For this review, take the finished solid that the model builds, in its own axes (mm). A direction names the side the tool comes from. Round coordinates to 2 decimals unless told otherwise and drop trailing zeros. Loops run counter-clockwise (first coordinate to the right, second up) from the corner with the lowest first, then second, coordinate; pieces in that order, holes last.
1. Consider section A-A on x = -55. State the section outline as (y, z) points.
2. Draft analysis for pull direction X (two halves, no side actions). For faces 6 (the flat face through (-20, 49, 14)), 7 (the flat face through (35, 47, 13)), 8 (the flat face through (-52, 25, 4)), 9 (the flat face through (20, 49, 14)), state which applies: released by +X, released by -X, zero draft, split by the parting line, or undercut.
3. To check wall thickness, follow line 1 along X through (y, z) = (45, 27); line 2 along Y through (x, z) = (-54, 14.5); line 3 along Y through (x, z) = (-6, -13.5). State the ranges of each line that lie inside material, in increasing order.
4. Tool access review of faces 1 (the flat face through (1, 0, -10)), 2 (the flat face through (-35, 47, 13)), 3 (the flat face through (-60, 12, -24.27)), 4 (the flat face through (57, 25, 4)), 5 (the cylindrical face through (0.77, 14.79, -73.26)): name each direction out of +Z, -Z, +X, -X, +Y, -Y from which nothing blocks a thin tool from reaching the whole face with its end or side.
5. Clearance check with flat-ended pins moving along their axes: pin 1 Ø12 at (y, z) = (64, 2) entering from -X; pin 2 Ø17 at (x, y) = (-63.5, 9) entering from -Z; pin 3 Ø17.5 at (x, z) = (55.5, 1.5) entering from +Y. State where each tip first meets the part, or that it passes through.
6. Consider section B-B on z = 5.5. State the section outline as (x, y) points, then the cut area to 3 significant figures.
7. Consider section D-D on z = -36. State the section outline as (x, y) points, then the cut area to 3 significant figures.
8. Consider section C-C on y = 44.5. State the section outline as (x, z) points.
from build123d import *

# Parameters (mm, degrees)
BASE_PLATE_DEPTH               = 25
HOUSING_PROFILE_CUT_DEPTH      = 61
HOUSING_PROFILE_CUT_DEPTH_BACK = 91
HOUSING_BOSS_DEPTH             = 5
BORE_40_DEPTH                  = 110
BORE_40_DEPTH_BACK             = 116
BORE_40_SKETCH_R               = 20
MOUNTING_HOLE_10_A_SKETCH_R    = 5
MOUNTING_HOLE_10_A_DEPTH       = 393
MOUNTING_HOLE_10_B_DEPTH       = 393
MOUNTING_HOLE_10_B_DEPTH_BACK  = 393
MOUNTING_HOLE_10_B_SKETCH_R    = 5
CLEVIS_LUGS_DEPTH              = 70
LUG_GAP_CUT_SKETCH_W           = 40
LUG_GAP_CUT_SKETCH_H           = 47
LUG_GAP_CUT_DEPTH              = 207
PIN_HOLE_10_DEPTH              = 207
PIN_HOLE_10_DEPTH_BACK         = 207
PIN_HOLE_10_SKETCH_R           = 5


with BuildPart() as part:
    # Base Plate Sketch → Base Plate (new body)
    with BuildSketch(Plane(origin=(0, 0, 0), x_dir=(1, 0, 0), z_dir=(0, 1, 0))):
        Polygon((-70, 95.100325632), (70, 95.100325632), (70, 73.269753582), (70, -31.730246418), (-70, -31.730246418), (-70, 73.269753582), align=None)
    extrude(amount=BASE_PLATE_DEPTH)

    # Housing Profile Cut Sketch → Housing Profile Cut (cut, two sides: drawn at the far end of the back side and taken through both)
    with BuildSketch(Plane(origin=(0, 25, 0), x_dir=(1, 0, 0), z_dir=(0, 1, 0)).offset(-HOUSING_PROFILE_CUT_DEPTH_BACK)):
        with BuildLine():
            Line((49, 24.269753582), (70, 24.269753582))
            Line((70, 24.269753582), (70, 95.100325632))
            Line((70, 95.100325632), (-70, 95.100325632))
            Line((-70, 95.100325632), (-70, 24.269753582))
            Line((-70, 24.269753582), (-49, 24.269753582))
            ThreePointArc((-49, 24.269753582), (-39.100505063, 28.370258646), (-35, 38.269753582))
            ThreePointArc((-35, 38.269753582), (0, 73.269753582), (35, 38.269753582))
            ThreePointArc((35, 38.269753582), (39.100505063, 28.370258646), (49, 24.269753582))
        make_face()
    extrude(amount=HOUSING_PROFILE_CUT_DEPTH + HOUSING_PROFILE_CUT_DEPTH_BACK, mode=Mode.SUBTRACT)

    # Housing Boss Sketch → Housing Boss (add)
    with BuildSketch(Plane(origin=(0, 25, 0), x_dir=(1, 0, 0), z_dir=(0, 1, 0))):
        with BuildLine():
            ThreePointArc((-35, 38.269753582), (0, 3.269753582), (35, 38.269753582))
            ThreePointArc((35, 38.269753582), (0, 73.269753582), (-35, 38.269753582))
        make_face()
        with BuildLine():
            Line((35, -31.730246418), (35, 38.269753582))
            ThreePointArc((35, 38.269753582), (0, 3.269753582), (-35, 38.269753582))
            Line((-35, 38.269753582), (-35, -31.730246418))
            Line((-35, -31.730246418), (35, -31.730246418))
        make_face()
    extrude(amount=HOUSING_BOSS_DEPTH)

    # Bore Ø40 Sketch → Bore Ø40 (cut, two sides: drawn at the far end of the back side and taken through both)
    with BuildSketch(Plane(origin=(0, 30, 0), x_dir=(1, 0, 0), z_dir=(0, 1, 0)).offset(-BORE_40_DEPTH_BACK)):
        with Locations(Location((0, 38.269753582, 0), (0, 0, 90))):
            Circle(BORE_40_SKETCH_R)
    extrude(amount=BORE_40_DEPTH + BORE_40_DEPTH_BACK, mode=Mode.SUBTRACT)

    # Mounting Hole Ø10 A Sketch → Mounting Hole Ø10 A (cut)
    with BuildSketch(Plane(origin=(0, 25, 0), x_dir=(1, 0, 0), z_dir=(0, 1, 0))):
        with Locations(Location((-55, -8.730246418, 0), (0, 0, 270))):
            Circle(MOUNTING_HOLE_10_A_SKETCH_R)
    extrude(amount=-MOUNTING_HOLE_10_A_DEPTH, mode=Mode.SUBTRACT)

    # Mounting Hole Ø10 B Sketch → Mounting Hole Ø10 B (cut, two sides: drawn at the far end of the back side and taken through both)
    with BuildSketch(Plane(origin=(0, 25, 0), x_dir=(1, 0, 0), z_dir=(0, 1, 0)).offset(-MOUNTING_HOLE_10_B_DEPTH_BACK)):
        with Locations(Location((51.913967656, -6.666465324, 0), (0, 0, 90))):
            Circle(MOUNTING_HOLE_10_B_SKETCH_R)
    extrude(amount=MOUNTING_HOLE_10_B_DEPTH + MOUNTING_HOLE_10_B_DEPTH_BACK, mode=Mode.SUBTRACT)

    # Clevis Lugs Sketch → Clevis Lugs (add)
    with BuildSketch(Plane(origin=(35, 0, 0), x_dir=(0, 0, -1), z_dir=(1, 0, 0))):
        with BuildLine():
            Line((-31.730246418, 65), (-31.730246418, 30))
            Line((-31.730246418, 30), (15.269753582, 30))
            Line((15.269753582, 30), (-3.026748887, 71.100340599))
            ThreePointArc((-3.026748887, 71.100340599), (-19.84854219, 79.67229469), (-31.730246418, 65))
        make_face()
    extrude(amount=-CLEVIS_LUGS_DEPTH)

    # Lug Gap Cut Sketch → Lug Gap Cut (cut)
    with BuildSketch(Plane(origin=(0, 30, 0), x_dir=(1, 0, 0), z_dir=(0, 1, 0))):
        with Locations((0, -8.230246418)):
            Rectangle(LUG_GAP_CUT_SKETCH_W, LUG_GAP_CUT_SKETCH_H)
    extrude(amount=LUG_GAP_CUT_DEPTH, mode=Mode.SUBTRACT)

    # Pin Hole Ø10 Sketch → Pin Hole Ø10 (cut, two sides: drawn at the far end of the back side and taken through both)
    with BuildSketch(Plane.ZY.offset(35).offset(-PIN_HOLE_10_DEPTH_BACK)):
        with Locations(Location((16.730246418, 65, 0), (0, 0, 180))):
            Circle(PIN_HOLE_10_SKETCH_R)
    extrude(amount=PIN_HOLE_10_DEPTH + PIN_HOLE_10_DEPTH_BACK, mode=Mode.SUBTRACT)


solid = part.part
Resolved:
1. outline: (0, -24.27) - (25, -24.27) - (25, 3.73) - (0, 3.73) - close; (0, 13.73) - (25, 13.73) - (25, 31.73) - (0, 31.73) - close
2. face 6: undercut
2. face 7: released by +X
2. face 8: zero draft
2. face 9: undercut
3. line 1: x = -35 to -20, 20 to 35
3. line 2: y = 0 to 25
3. line 3: y = 0 to 30
4. face 1: +Z, -Z, +X, -X, -Y
4. face 2: +Z, -Z, -X, +Y
4. face 3: -Z, -X, +Y, -Y
4. face 4: +Z, -Z, +X, +Y
4. face 5: -Z, +Y, -Y
5. pin 1: stops at x = -35
5. pin 2: stops at z = -24.27
5. pin 3: stops at y = 25
6. outline: (-70, 0) - (-58.82, 0) - (-58.82, 25) - (-70, 25) - close; (-51.18, 0) - (47.05, 0) - (47.05, 25) - (35, 25) - (35, 74.94) - (20, 74.94) - (20, 30) - (-20, 30) - (-20, 74.94) - (-35, 74.94) - (-35, 25) - (-51.18, 25) - close; (56.78, 0) - (70, 0) - (70, 25) - (56.78, 25) - close
6. area: 4,760 mm2
7. outline: (-35.19, 0) - (-19.87, 0) - (-19.87, 30) - (-35, 30) - (-35, 25) - (-35.19, 25) - close; (19.87, 0) - (35.19, 0) - (35.19, 25) - (35, 25) - (35, 30) - (19.87, 30) - close
7. area: 917 mm2
8. outline: (-35, -8.81) - (-20, -8.81) - (-20, 31.73) - (-35, 31.73) - close; (20, -8.81) - (35, -8.81) - (35, 31.73) - (20, 31.73) - close
